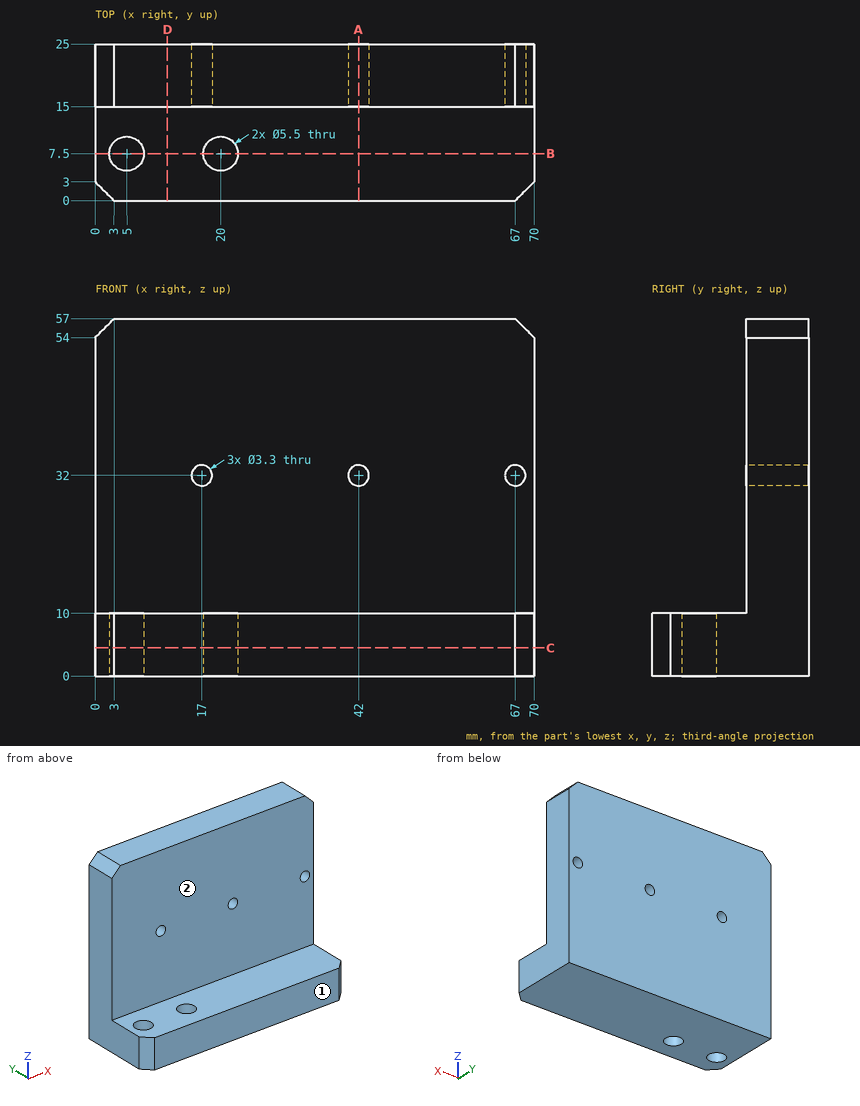
Source: three-view drawing plus pictorial views. Frame: mm from the lowest corner of the part. A direction names the side the tool comes from. Round coordinates to 2 decimals unless told otherwise and drop trailing zeros. Loops run counter-clockwise (first coordinate to the right, second up) from the corner with the lowest first, then second, coordinate; pieces in that order, holes last. Notation, with made-up numbers: M 51.5,4 L 71.5,4 A32 cw 71.5,35 Z; hole C -15.5,-22 d4. An arc over 180 degrees is marked long. Answer as CSV lines item,"result". Start each with the question number.
(1) Reachability of the marked faces 1 and 2 from +Z, -Z, +X, -X, +Y, -Y: full face, straight path, thin tool, end or side. Return the list, or none.
(2) Section A-A, the plane x = 42. Output: boundary loops of the cut face in (y, z), plus the area to 3 significant figures.
(3) First-contact query: pin 1 (2 mm diameter, centred on x = 19.5, y = 4.5, fed in from -Z); pin 2 (9 mm diameter, centred on x = 5, y = 7.5, fed in from +Z); pin 3 (4 mm diameter, centred on x = 67, z = 32, fed in from -Y). Flat tips, straight axial feed; report the tip coordinate or a pass-through.
(4) Line query: line 1 (X direction, y = 21, z = 32); line 2 (Z direction, x = 67, y = 20); line 3 (Y direction, x = 20, z = 6). Output: solid intervals per line, ascending. Write a range as [from, to].
(5) Section B-B, the plane y = 7.5. Output: boundary loops of the cut face in (x, z), plus the area to 3 significant figures.
(6) Section C-C, the plane z = 4.5. Output: boundary loops of the cut face in (x, y), plus the area to 3 significant figures.
(7) Section D-D, the plane x = 11.5. Output: boundary loops of the cut face in (y, z).
Values found:
1,face 1,"+Z, -Z, +X, -X, -Y"
1,face 2,"+Z, +X, -X, -Y"
2,outline,"M 0,0 L 25,0 L 25,30.35 L 15,30.35 L 15,10 L 0,10 Z; M 15,33.65 L 25,33.65 L 25,57 L 15,57 Z"
2,area,"687 mm²"
3,pin 1,"stops at z = 0"
3,pin 2,"stops at z = 10"
3,pin 3,"stops at y = 15"
4,line 1,"x = [0, 15.35], [18.65, 40.35], [43.65, 65.35], [68.65, 70]"
4,line 2,"z = [0, 30.35], [33.65, 57]"
4,line 3,"y = [0, 4.75], [10.25, 25]"
5,outline,"M 0,0 L 2.25,0 L 2.25,10 L 0,10 Z; M 7.75,0 L 17.25,0 L 17.25,10 L 7.75,10 Z; M 22.75,0 L 70,0 L 70,10 L 22.75,10 Z"
5,area,"590 mm²"
6,outline,"M 0,3 L 3,0 L 67,0 L 70,3 L 70,25 L 0,25 Z; hole C 5,7.5 d5.5; hole C 20,7.5 d5.5"
6,area,"1,690 mm²"
7,outline,"M 0,0 L 25,0 L 25,57 L 15,57 L 15,10 L 0,10 Z"
